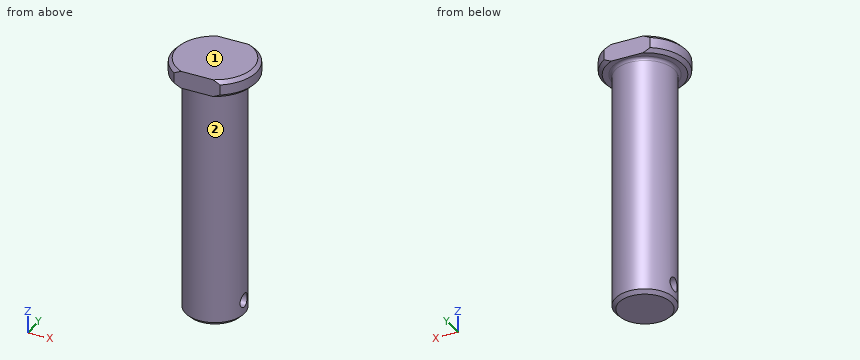
```python
from build123d import *

# Parameters (mm, degrees)
SKETCH2_R          = 2
CUT_EXTRUDE1_DEPTH = 10
SKETCH3_W          = 27.306431106
SKETCH3_H          = 8.074180861
SKETCH3_W_2        = 26.857865503
SKETCH3_H_2        = 8.130251561
CUT_EXTRUDE2_DEPTH = 5
FILLET1_R          = 0.8


with BuildPart() as part:
    # Sketch1 → Revolve1 (revolve)
    with BuildSketch(Plane(origin=(0, 0, 0), x_dir=(0, 0, -1), z_dir=(1, 0, 0)), mode=Mode.PRIVATE) as revolve1_sk:
        Polygon((5, 8.5), (5, 0), (75, 0), (75, 7.5), (74, 8.5), align=None)
        Polygon((4, 12), (5, 11), (5, 0), (0, 0), (0, 11), (1, 12), align=None)
    revolve(revolve1_sk.sketch.rotate(Axis((0, 0, -5), (0, 0, -1)), 90), axis=Axis((0, 0, -5), (0, 0, -1)))

    # Sketch2 → Cut-Extrude1 (cut, symmetric)
    with BuildSketch(Plane(origin=(0, 0, 0), x_dir=(0, 0, -1), z_dir=(1, 0, 0))):
        with Locations((70, 0)):
            Circle(SKETCH2_R)
    extrude(amount=CUT_EXTRUDE1_DEPTH, both=True, mode=Mode.SUBTRACT)

    # Sketch3 → Cut-Extrude2 (cut, symmetric)
    with BuildSketch(Plane.XY):
        with Locations((-0.627385884, 14.037090431)):
            Rectangle(SKETCH3_W, SKETCH3_H)
        with Locations((0.662240226, -14.065125781)):
            Rectangle(SKETCH3_W_2, SKETCH3_H_2)
    extrude(amount=CUT_EXTRUDE2_DEPTH, both=True, mode=Mode.SUBTRACT)

    # Fillet1
    fillet1_edges = [part.edges().sort_by_distance(p)[0] for p in [
        (-8.5, 0, -5),
    ]]
    fillet(fillet1_edges, radius=FILLET1_R)


solid = part.part
```
Geometry check sheet. Reference: the model listing, model coordinates, mm. Face numbers are marked on the shaded views. A direction names the side the tool comes from. Give positions to 0.01 mm unless a question says otherwise; leave off trailing zeros. Order: outer loops, then holes, each group sorted by start corner. A loop starts at its lowest first (then second) coordinate and runs counter-clockwise, first axis right, second up. Notation, with made-up numbers: (35, 75) - (65, 75) arc R24 cw to (65, 111) - close; hole circle Ø8 at (36, 34.25). An arc over 180 degrees is marked (long way). Write item = value, one per line. Start each with the question number.
1) Section check B-B (x = 0). Enter the section's corners in (y, z), then the cut area to 3 significant figures.
2) Gauge pin test, flat ends, axial feed: pin 1 Ø2 at (y, z) = (-3, -31) entering from +X; pin 2 Ø12 at (y, z) = (-0.5, -49) entering from -X; pin 3 Ø6 at (x, z) = (5, -30.5) entering from +Y. Record the tip position at first contact, or that the pin passes through.
3) Section check C-C (z = -70). Enter the section's corners in (x, y), then the cut area to 3 significant figures.
4) Section check A-A (y = 0). Enter the section's corners in (x, z).
5) Scan lines: L1, parallel to Z at x = -4.5, y = 0; L2, parallel to Y at x = 0.25, z = -70; L3, parallel to Z at x = 7, y = -7.25. Record each from-to range of solid material in increasing order.
6) Access from +Z, -Z, +X, -X, +Y, -Y to the whole of each face (thin tool, end or side, straight path). Record for the marked faces 1 and 2.
Geometry check:
q1.outline = (-10, -5) - (-9.3, -5) arc R0.8 cw to (-8.5, -5.8) - (-8.5, -74) - (-7.5, -75) - (7.5, -75) - (8.5, -74) - (8.5, -5.8) arc R0.8 cw to (9.3, -5) - (10, -5) - (10, 0) - (-10, 0) - close; hole circle Ø4 at (0, -70)
q1.area = 1,280 mm2
q2.pin_1 = 8.26
q2.pin_2 = -8.5
q2.pin_3 = 8.26
q3.outline = (-8.26, -2) arc R8.5 ccw to (8.26, -2) - close; (-8.26, 2) - (8.26, 2) arc R8.5 ccw to start
q3.area = 160 mm2
q4.outline = (-12, -4) - (-11, -5) - (-9.3, -5) arc R0.8 cw to (-8.5, -5.8) - (-8.5, -68) - (8.5, -68) - (8.5, -5.8) arc R0.8 cw to (9.3, -5) - (11, -5) - (12, -4) - (12, -1) - (11, 0) - (-11, 0) - (-12, -1) - close; (-8.5, -74) - (-7.5, -75) - (7.5, -75) - (8.5, -74) - (8.5, -72) - (-8.5, -72) - close
q5.L1 = -75 to -72, -68 to 0
q5.L2 = -8.5 to -2, 2 to 8.5
q5.L3 = -5 to 0
q6.face_1 = +Z, +X, -X, +Y, -Y
q6.face_2 = -Z
